For this review, take the finished solid that the model builds, in its own axes (mm). Face numbers are marked on the shaded views. A direction names the side the tool comes from. Give positions to 0.01 mm unless a question says otherwise; leave off trailing zeros. Write each loop counter-clockwise with the first axis right and the second up, starting at its lowest first coordinate (ties: lowest second). Pieces come first, ordered by that corner, then holes. Notation, with made-up numbers: M 20,80 L 37,80 A21 ccw 37,102 Z; hole C -19,-23.5 d11. An arc over 180 degrees is marked long. Answer as a JSON object with one key per item and string values. Group by question number.
```python
from build123d import *

# Parameters (mm, degrees)
BASE_BLOCK_SKETCH_W       = 36
BASE_BLOCK_SKETCH_H       = 29
BASE_BLOCK_DEPTH          = 24
OFFSET_ARM_DEPTH          = 15
ARM_RISER_DEPTH           = 18
UPPER_ARM_SKETCH_W        = 15
UPPER_ARM_SKETCH_H        = 11
UPPER_ARM_DEPTH           = 18
PIVOT_LUG_DEPTH           = 15
PIVOT_HOLE_SKETCH_R       = 4.5
PIVOT_HOLE_DEPTH          = 15
CLAMP_BODY_DEPTH          = 29
CLAMP_JAW_SKETCH_W        = 29
CLAMP_JAW_SKETCH_H        = 44
CLAMP_JAW_DEPTH           = 12
CLAMP_JAW_END_DEPTH       = 12
CLAMP_BORE_AND_SLOT_DEPTH = 12
WINDOW_SKETCH_W           = 24
WINDOW_SKETCH_H           = 12
RECTANGULAR_WINDOW_DEPTH  = 50
CROSS_HOLE_SKETCH_R       = 3
CLAMP_CROSS_HOLE_DEPTH    = 50


with BuildPart() as part:
    # Base Block Sketch → Base Block (new body)
    with BuildSketch(Plane.XY):
        with Locations((18, -14.5)):
            Rectangle(BASE_BLOCK_SKETCH_W, BASE_BLOCK_SKETCH_H)
    extrude(amount=BASE_BLOCK_DEPTH)

    # Offset Arm Sketch → Offset Arm (add)
    with BuildSketch(Plane.XY.offset(24)):
        with BuildLine():
            Line((0, -29), (-24, -29))
            ThreePointArc((-24, -29), (-36.727922061, -23.727922061), (-42, -11))
            Line((-42, -11), (-42, -6))
            Line((-42, -6), (-41.291616466, -6))
            Line((-41.291616466, -6), (-24, -6))
            Line((-24, -6), (-24, -11))
            Line((-24, -11), (0, -11))
            Line((0, -11), (0, -29))
        make_face()
    extrude(amount=-OFFSET_ARM_DEPTH)

    # Arm Riser Sketch → Arm Riser (add)
    with BuildSketch(Plane.ZY.offset(42)):
        Polygon((-9, 17), (9, -6), (24, -6), (6, 17), align=None)
    extrude(amount=-ARM_RISER_DEPTH)

    # Upper Arm Sketch → Upper Arm (add)
    with BuildSketch(Plane.ZY.offset(42)):
        with Locations((-1.5, 22.5)):
            Rectangle(UPPER_ARM_SKETCH_W, UPPER_ARM_SKETCH_H)
    extrude(amount=-UPPER_ARM_DEPTH)

    # Pivot Lug Sketch → Pivot Lug (add)
    with BuildSketch(Plane.XY.offset(6)):
        with BuildLine():
            Line((-42, 28), (-24, 28))
            ThreePointArc((-24, 28), (-33, 37), (-42, 28))
        make_face()
    extrude(amount=-PIVOT_LUG_DEPTH)

    # Pivot Hole Sketch → Pivot Hole (cut)
    with BuildSketch(Plane.XY.offset(6)):
        with Locations((-33, 28)):
            Circle(PIVOT_HOLE_SKETCH_R)
    extrude(amount=-PIVOT_HOLE_DEPTH, mode=Mode.SUBTRACT)

    # Clamp Body Sketch → Clamp Body (add)
    with BuildSketch(Plane(origin=(0, 0, 0), x_dir=(1, 0, 0), z_dir=(0, 1, 0))):
        Polygon((36, -6), (36, -12), (36, -18), (48, -18), (48, -6), align=None)
    extrude(amount=-CLAMP_BODY_DEPTH)



with BuildPart() as body_2:
    # Clamp Jaw Sketch → Clamp Jaw (new body)
    with BuildSketch(Plane.XY.offset(18)):
        with Locations((62.5, 22)):
            Rectangle(CLAMP_JAW_SKETCH_W, CLAMP_JAW_SKETCH_H)
    extrude(amount=-CLAMP_JAW_DEPTH)


with BuildPart() as part_1:
    add(part.part)

    add(body_2.part)  # Clamp Jaw End merges body 2
    # Clamp Jaw End Sketch → Clamp Jaw End (add)
    with BuildSketch(Plane.XY.offset(18)):
        with BuildLine():
            Line((48, 0), (77, 0))
            ThreePointArc((77, 0), (68.506096654, -20.506096654), (48, -29))
            Line((48, -29), (48, 0))
        make_face()
    extrude(amount=-CLAMP_JAW_END_DEPTH)

    # Clamp Bore Slot Sketch → Clamp Bore and Slot (cut)
    with BuildSketch(Plane.XY.offset(18)):
        with BuildLine():
            Line((62.5, 44), (61.5, 44))
            Line((61.5, 44), (61.5, 26.92820323))
            ThreePointArc((61.5, 26.92820323), (62.5, 13), (63.5, 26.92820323))
            Line((63.5, 26.92820323), (63.5, 44))
            Line((63.5, 44), (62.5, 44))
        make_face()
    extrude(amount=-CLAMP_BORE_AND_SLOT_DEPTH, mode=Mode.SUBTRACT)

    # Window Sketch → Rectangular Window (cut)
    with BuildSketch(Plane(origin=(0, 0, 0), x_dir=(1, 0, 0), z_dir=(0, 1, 0))):
        with Locations((18, -12)):
            Rectangle(WINDOW_SKETCH_W, WINDOW_SKETCH_H)
    extrude(amount=-RECTANGULAR_WINDOW_DEPTH, mode=Mode.SUBTRACT)

    # Cross Hole Sketch → Clamp Cross Hole (cut)
    with BuildSketch(Plane.ZY.offset(-48)):
        with Locations((12, 38)):
            Circle(CROSS_HOLE_SKETCH_R)
    extrude(amount=-CLAMP_CROSS_HOLE_DEPTH, mode=Mode.SUBTRACT)


solid = part_1.part
```
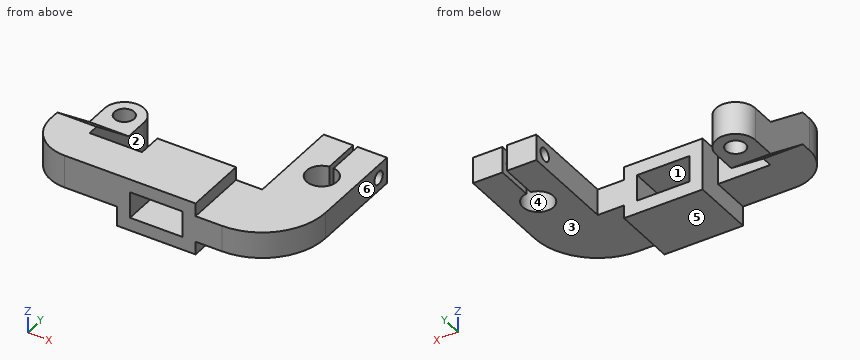
Item 1: Consider section D-D (x = 59.5). Give the boundary of the cut face in (y, z), plus the area to 3 significant figures.
Item 2: Draft analysis for pull direction X (two halves, no side actions). For the marked faces 4, 5 and 6, state which applies: released by +X, released by -X, zero draft, split by the parting line, or undercut.
Item 3: Consider section C-C (z = 12). Give the boundary of the cut face in (x, y), plus the area to 4 significant figures.
Item 4: To check wall thickness, follow probe 1 along X at (y, z) = (20, 11.25); probe 2 along Z at (x, y) = (13, -25); probe 3 along Y at (x, z) = (67, 12). State the ranges of each line that lie inside material, in increasing order.
Item 5: Consider section B-B (y = 20). Give the boundary of the cut face in (x, z).
Item 6: Consider section A-A (x = 22). Give the boundary of the cut face in (y, z).
Item 7: Insertion check: P1, Ø1.5, axis at x = 12.5, z = 15.5, coming from the +Y side; P2, Ø1.8, axis at y = -9, z = 21.5, coming from the +X side; P3, Ø3.5, axis at y = 36.5, z = 12, coming from the -X side; P4, Ø2, axis at y = -17, z = 0.5, coming from the -X side. Each pin has a flat end and moves straight along its axis. Give the tip position at first contact, or say it passes through.
Item 8: Machinability: for the marked faces 1, 2 and 3, which of the approach directions +Z, -Z, +X, -X, +Y, -Y give a long, thin tool a straight path to every point of the face, cutting with its end or side? Answer none if there is none.
Result set:
{
 "1": {"outline": "M -26.62,6 L 13.68,6 L 13.68,18 L -26.62,18 Z; M 26.32,6 L 44,6 L 44,18 L 26.32,18 Z; hole C 38,12 d6", "area": "667 mm^2"},
 "2": {"face 4": "undercut", "face 5": "zero draft", "face 6": "released by +X"},
 "3": {"outline": "M -42,-11 A18 ccw -24,-29 L 6,-29 L 6,0 L 0,0 L 0,-11 L -24,-11 L -24,9.33 L -42,9.33 Z; M 30,-29 L 48,-29 A29 ccw 77,0 L 77,35 L 63.5,35 L 63.5,26.93 A7 cw long 61.5,26.93 L 61.5,35 L 48,35 L 48,0 L 30,0 Z; M 48,41 L 61.5,41 L 61.5,44 L 48,44 Z; M 63.5,41 L 77,41 L 77,44 L 63.5,44 Z", "area": "3,335 mm^2"},
 "4": {"probe 1": "x = 48 to 55.5, 69.5 to 77", "probe 2": "z = 0 to 6, 18 to 24", "probe 3": "y = -21.91 to 14.64, 25.36 to 35, 41 to 44"},
 "5": {"outline": "M -42,-9 L -24,-9 L -24,6 L -42,6 Z; M 48,6 L 55.5,6 L 55.5,18 L 48,18 Z; M 69.5,6 L 77,6 L 77,18 L 69.5,18 Z"},
 "6": {"outline": "M -29,0 L 0,0 L 0,6 L -29,6 Z; M -29,18 L 0,18 L 0,24 L -29,24 Z"},
 "7": {"P1": "passes through", "P2": "stops at x = 36", "P3": "stops at x = 48", "P4": "stops at x = 0"},
 "8": {"face 1": "+Y, -Y", "face 2": "+Z, -Z, +Y", "face 3": "-Z, +X, +Y, -Y"}
}
